Verification items for the finished model (mm, model axes). Face numbers are marked on the shaded views. A direction names the side the tool comes from. Round coordinates to 2 decimals unless told otherwise and drop trailing zeros. Loops run counter-clockwise (first coordinate to the right, second up) from the corner with the lowest first, then second, coordinate; pieces in that order, holes last. Notation, with made-up numbers: (-17, 83.25) - (39, 83.25) arc R19 cw to (39, 111.25) - close; hole circle Ø5 at (1.25, 9.5). An arc over 180 degrees is marked (long way). Use CSV: the item, a comma, the result in double quotes.
```python
from build123d import *

# Parameters (mm, degrees)
SKETCH1_W             = 90
SKETCH1_H             = 70
BOSS_EXTRUDE1_DEPTH   = 35
SKETCH2_W             = 80
SKETCH2_H             = 60
CUT_EXTRUDE1_DEPTH    = 33
FILLET1_R             = 5
M3_TAPPED_HOLE1_D     = 2.5
M3_TAPPED_HOLE1_DEPTH = 8.5
M3_TAPPED_HOLE1_TIP   = 0.751075774
SKETCH7_R             = 4
CUT_EXTRUDE2_DEPTH    = 10


with BuildPart() as part:
    # Sketch1 → Boss-Extrude1 (new body)
    with BuildSketch(Plane(origin=(0, 0, 0), x_dir=(1, 0, 0), z_dir=(0, 1, 0))):
        Rectangle(SKETCH1_W, SKETCH1_H)
    extrude(amount=BOSS_EXTRUDE1_DEPTH)

    # Sketch2 → Cut-Extrude1 (cut)
    with BuildSketch(Plane(origin=(0, 35, 0), x_dir=(1, 0, 0), z_dir=(0, 1, 0))):
        Rectangle(SKETCH2_W, SKETCH2_H)
    extrude(amount=-CUT_EXTRUDE1_DEPTH, mode=Mode.SUBTRACT)

    # Fillet1
    fillet1_edges = [part.edges().sort_by_distance(p)[0] for p in [
        (40, 18.5, -30),
        (40, 18.5, 30),
        (-40, 18.5, 30),
        (-40, 18.5, -30),
        (45, 17.5, 35),
        (-45, 17.5, 35),
        (-45, 17.5, -35),
        (45, 17.5, -35),
    ]]
    fillet(fillet1_edges, radius=FILLET1_R)

    # M3 Tapped Hole1
    with Locations(Plane(origin=(0, 35, 0), x_dir=(1, 0, 0), z_dir=(0, 1, 0))):
        with Locations((-41, 31), (41, 31), (41, -31), (-41, -31)):
            Hole(M3_TAPPED_HOLE1_D / 2, depth=M3_TAPPED_HOLE1_DEPTH)
            with Locations((0, 0, -(M3_TAPPED_HOLE1_DEPTH + M3_TAPPED_HOLE1_TIP / 2))):  # 118° drill point
                Cone(0, M3_TAPPED_HOLE1_D / 2, M3_TAPPED_HOLE1_TIP, mode=Mode.SUBTRACT)

    # Sketch7 → Cut-Extrude2 (cut)
    with BuildSketch(Plane.ZY.offset(45)):
        with Locations((-16.5, 22.4)):
            Circle(SKETCH7_R)
    extrude(amount=-CUT_EXTRUDE2_DEPTH, mode=Mode.SUBTRACT)


solid = part.part
```
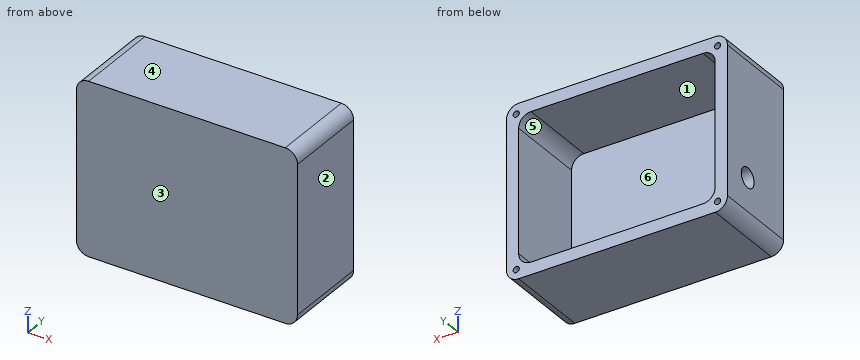
1) Cross-section at C-C, the plane x = -3. Record the cut outline in (y, z), then the cut area to 3 significant figures.
Returned:
outline,"(0, -35) - (35, -35) - (35, -30) - (2, -30) - (2, 30) - (35, 30) - (35, 35) - (0, 35) - close"
area,"470 mm²"
2) Cross-section at D-D, the plane y = 28. Record the cut outline in (x, z), then the cut area to 3 significant figures.
Returned:
outline,"(-45, -30) arc R5 ccw to (-40, -35) - (40, -35) arc R5 ccw to (45, -30) - (45, 30) arc R5 ccw to (40, 35) - (-40, 35) arc R5 ccw to (-45, 30) - close; hole circle Ø2.5 at (-41, -31); hole circle Ø2.5 at (-41, 31); hole (-40, -25) arc R5 ccw to (-35, -30) - (35, -30) arc R5 ccw to (40, -25) - (40, 25) arc R5 ccw to (35, 30) - (-35, 30) arc R5 ccw to (-40, 25) - close; hole circle Ø2.5 at (41, -31); hole circle Ø2.5 at (41, 31)"
area,"1,480 mm²"
3) Cross-section at B-B, the plane y = 4.5. Record the cut outline in (x, z), then the cut area to 3 significant figures.
Returned:
outline,"(-45, -30) arc R5 ccw to (-40, -35) - (40, -35) arc R5 ccw to (45, -30) - (45, 30) arc R5 ccw to (40, 35) - (-40, 35) arc R5 ccw to (-45, 30) - close; hole (-40, -25) arc R5 ccw to (-35, -30) - (35, -30) arc R5 ccw to (40, -25) - (40, 25) arc R5 ccw to (35, 30) - (-35, 30) arc R5 ccw to (-40, 25) - close"
area,"1,500 mm²"
4) Gauge pin test, flat ends, axial feed: pin 1 Ø4 at (x, z) = (14, -1) entering from +Y; pin 2 Ø2 at (x, z) = (-41, -31) entering from +Y; pin 3 Ø5 at (y, z) = (22.4, -16.5) entering from -X; pin 4 Ø3 at (x, z) = (41, -31) entering from -Y. Record the tip position at first contact, or that the pin passes through.
Returned:
pin 1,"stops at y = 2"
pin 2,"stops at y = 26.35"
pin 3,"stops at x = 40"
pin 4,"stops at y = 0"
5) Thickness scan on probe 1 along X at (y, z) = (5, -7); probe 2 along Z at (x, y) = (12, 3); probe 3 along Z at (x, y) = (-41, 29). Record the ranges inside material, lowest first. Write a range as [from, to].
Returned:
probe 1,"x = [-45, -40], [40, 45]"
probe 2,"z = [-35, -30], [30, 35]"
probe 3,"z = [-34.9, -32.25], [-29.75, 29.75], [32.25, 34.9]"
6) Mould release check, pull along Z, two halves, no side actions. Record for the marked faces 3, 4, 5 and 6: +Z half, -Z half, draft (parallel to the pull), parting line (faces both ways), or undercut.
Returned:
face 3,"draft"
face 4,"+Z half"
face 5,"undercut"
face 6,"undercut"
7) Cross-section at A-A, the plane z = -16.5. Record the cut outline in (x, y).
Returned:
outline,"(-45, 0) - (45, 0) - (45, 35) - (40, 35) - (40, 2) - (-40, 2) - (-40, 18.4) - (-45, 18.4) - close; (-45, 26.4) - (-40, 26.4) - (-40, 35) - (-45, 35) - close"
8) Access from +Z, -Z, +X, -X, +Y, -Y to the whole of each face (thin tool, end or side, straight path). Record for the marked faces 1 and 2.
Returned:
face 1,"+Y"
face 2,"+Z, -Z, +X, +Y, -Y"
